Read the model definition and answer for the solid it produces. Units are mm, in the model's axes. Face numbers are marked on the shaded views. A direction names the side the tool comes from. Coordinates: 2 decimals unless noted, no trailing zeros. Write each loop counter-clockwise with the first axis right and the second up, starting at its lowest first coordinate (ties: lowest second). Pieces come first, ordered by that corner, then holes.
1) The part is cut by section B-B (y = -2.5). Determine the outline of the cut face in (x, z).
2) The part is cut by section A-A (x = 10). Determine the outline of the cut face in (y, z).
3) The part is cut by section D-D (x = 6). Determine the outline of the cut face in (y, z), then the cut area to 3 significant figures.
4) Find the intervals of material crossed by line 1 (Z direction, x = 17, y = -6.75); line 2 (Y direction, x = 16, z = -15); line 3 (X direction, y = 4.25, z = -24), in increasing order.
5) Which of the six approach directions +Z, -Z, +X, -X, +Y, -Y give full straight-line access (tool end or side, diameter ignored) to the marked faces 1 and 2?
6) Each of these flat-tipped pins is pushed along its axis until it touches: pin 1 Ø1.5 at (y, z) = (4.5, -21) entering from +X; pin 2 Ø1 at (x, z) = (24, -19.5) entering from -Y; pin 3 Ø1.5 at (x, y) = (20, -8.5) entering from -Z. Where does it stop, or does it pass through?
7) Determine the mould class of the marked faces 3, 4 and 5 for opening direction X: +X half, -X half, draft (parallel to the pull), parting line (faces both ways), or undercut.
8) The part is cut by section C-C (z = -25). Determine the outline of the cut face in (x, y), then the cut area to 3 significant figures.
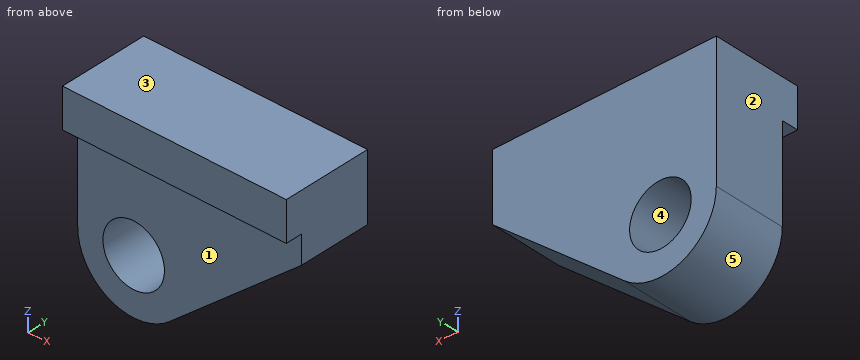
from build123d import *

# Parameters (mm, degrees)
SKETCH1_R           = 5.5
BOSS_EXTRUDE1_DEPTH = 6.5
SKETCH2_W           = 40
SKETCH2_H           = 7
BOSS_EXTRUDE2_DEPTH = 3


with BuildPart() as part:
    # Sketch1 → Boss-Extrude1 (new, symmetric)
    with BuildSketch(Plane(origin=(0, 0, 0), x_dir=(1, 0, 0), z_dir=(0, 1, 0))):
        with BuildLine():
            Line((40, 12), (16.405124482, 31.679477871))
            ThreePointArc((16.405124482, 31.679477871), (5.760380018, 33.056799788), (0, 24))
            Line((0, 24), (0, 0))
            Line((0, 0), (40, 0))
            Line((40, 0), (40, 12))
        make_face()
        with Locations(Location((10, 24, 0), (0, 0, 90))):
            Circle(SKETCH1_R, mode=Mode.SUBTRACT)
    extrude(amount=BOSS_EXTRUDE1_DEPTH, both=True)

    # Sketch2 → Boss-Extrude2 (add)
    with BuildSketch(Plane(origin=(0, -6.5, 0), x_dir=(1, 0, 0), z_dir=(0, 1, 0))):
        with Locations((20, 3.5)):
            Rectangle(SKETCH2_W, SKETCH2_H)
    extrude(amount=-BOSS_EXTRUDE2_DEPTH)


solid = part.part
Reported:
1. outline: (0, -24) arc R10 ccw to (16.41, -31.68) - (40, -12) - (40, 0) - (0, 0) - close; hole circle Ø11 at (10, -24)
2. outline: (-9.5, -7) - (-6.5, -7) - (-6.5, -18.5) - (6.5, -18.5) - (6.5, 0) - (-9.5, 0) - close; (-6.5, -34) - (6.5, -34) - (6.5, -29.5) - (-6.5, -29.5) - close
3. outline: (-9.5, -7) - (-6.5, -7) - (-6.5, -20.23) - (6.5, -20.23) - (6.5, 0) - (-9.5, 0) - close; (-6.5, -33.17) - (6.5, -33.17) - (6.5, -27.77) - (-6.5, -27.77) - close
3. area: 354 mm2
4. line 1: z = -7 to 0
4. line 2: y = -6.5 to 6.5
4. line 3: x = 0 to 4.5, 15.5 to 25.61
5. face 1: -Z, +X, -X, -Y
5. face 2: +Z, -Z, -X, +Y, -Y
6. pin 1: stops at x = 30.11
6. pin 2: stops at y = -6.5
6. pin 3: stops at z = -7
7. face 3: draft
7. face 4: undercut
7. face 5: parting line
8. outline: (0.05, -6.5) - (4.59, -6.5) - (4.59, 6.5) - (0.05, 6.5) - close; (15.41, -6.5) - (24.41, -6.5) - (24.41, 6.5) - (15.41, 6.5) - close
8. area: 176 mm2
